CAD build for the part. Positions are in the model's coordinates, mm. A direction names the side the tool comes from. Round coordinates to 2 decimals unless told otherwise and drop trailing zeros. Order: outer loops, then holes, each group sorted by start corner. A loop starts at its lowest first (then second) coordinate and runs counter-clockwise, first axis right, second up. Notation, with made-up numbers: (-26, 29.25) -> (-22, 29.25) arc R24 ccw to (-22, 51.25) -> close; hole circle Ø6 at (72.5, 14.5). An arc over 180 degrees is marked (long way). Return JSON: item names as keys, results as strings. Group by question number.
Q1. Flat gauge pins, fed straight in: pin 1 (3 mm diameter, centred on x = 37.5, z = 1, fed in from -Y); pin 2 (5 mm diameter, centred on x = 20.5, z = -1, fed in from +Y); pin 3 (1.1 mm diameter, centred on y = -1, z = -1.5, fed in from -X); pin 4 (2 mm diameter, centred on x = 31.5, z = 3, fed in from +Y). Where does each tip first touch, or does it go through?
Q2. Probe line 1 along X through (y, z) = (-3.5, -0.75); line 2 along Z through (x, y) = (40, 1.5); line 3 along Y through (x, z) = (19, 0). List the from-to ranges inside material, lowest first.
Q3. Mould opens along Y. For faces 4 (the cylindrical face through (22.57, -2.44, -0.54)), 5 (the flat face through (45, 0, 0)), 6 (the flat face through (-3.77, -1.74, -0.99)) say: +Y half, -Y half, draft (parallel to the pull), parting line (faces both ways), or undercut.
Q4. Which spindle directions (+Z, -Z, +X, -X, +Y, -Y) get a long thin tool onto all of the face, cutting with end or side? Do faces 1 (the flat face through (-5, -2, -2)), 2 (the flat face through (-4, 0, -2)), 3 (the flat face through (0, -2, 2)). Say none if no direction does.
Q5. Cut at A-A (x = 6). Write the cut outline in (y, z).
from build123d import *

# Parameters (mm, degrees)
CUT_EXTRUDE1_DEPTH = 2.5


with BuildPart() as part:
    # Sketch1 → Revolve1 (revolve)
    with BuildSketch(Plane.XY, mode=Mode.PRIVATE) as revolve1_sk:
        Polygon((-5, 0), (-5, 3.683333333), (-4.433333333, 4.25), (0, 4.25), (0, 2.5), (44.508532, 2.5), (45, 2.008532), (45, 0), align=None)
    revolve(revolve1_sk.sketch.rotate(Axis((45, 0, 0), (-1, 0, 0)), 270), axis=Axis((45, 0, 0), (-1, 0, 0)))

    # Sketch2 → Cut-Revolve1 (revolve, cut)
    with BuildSketch(Plane.XY, mode=Mode.PRIVATE) as cut_revolve1_sk:
        Polygon((-5, 0), (-5, 2), (-2.5, 2), (-1.964101615, 0), align=None)
    revolve(cut_revolve1_sk.sketch.rotate(Axis((-1.964101615, 0, 0), (-1, 0, 0)), 270), axis=Axis((-1.964101615, 0, 0), (-1, 0, 0)), mode=Mode.SUBTRACT)

    # Sketch3 → Cut-Extrude1 (cut)
    with BuildSketch(Plane(origin=(-5, 0, 0), x_dir=(0, 0, -1), z_dir=(1, 0, 0))):
        Polygon((-2, 1.154700538), (-2, -1.154700538), (0, -2.309401077), (2, -1.154700538), (2, 1.154700538), (0, 2.309401077), align=None)
    extrude(amount=CUT_EXTRUDE1_DEPTH, mode=Mode.SUBTRACT)


solid = part.part
Solution:
{
 "1": {"pin 1": "stops at y = -2.5", "pin 2": "stops at y = 2.5", "pin 3": "stops at x = -5", "pin 4": "stops at y = 1.5"},
 "2": {"line 1": "x = -5 to 0", "line 2": "z = -2 to 2", "line 3": "y = -2.5 to 2.5"},
 "3": {"face 4": "parting line", "face 5": "draft", "face 6": "undercut"},
 "4": {"face 1": "+Z, -Z, -X, +Y, -Y", "face 2": "-X", "face 3": "+X"},
 "5": {"outline": "circle Ø5 at (0, 0)"}
}
